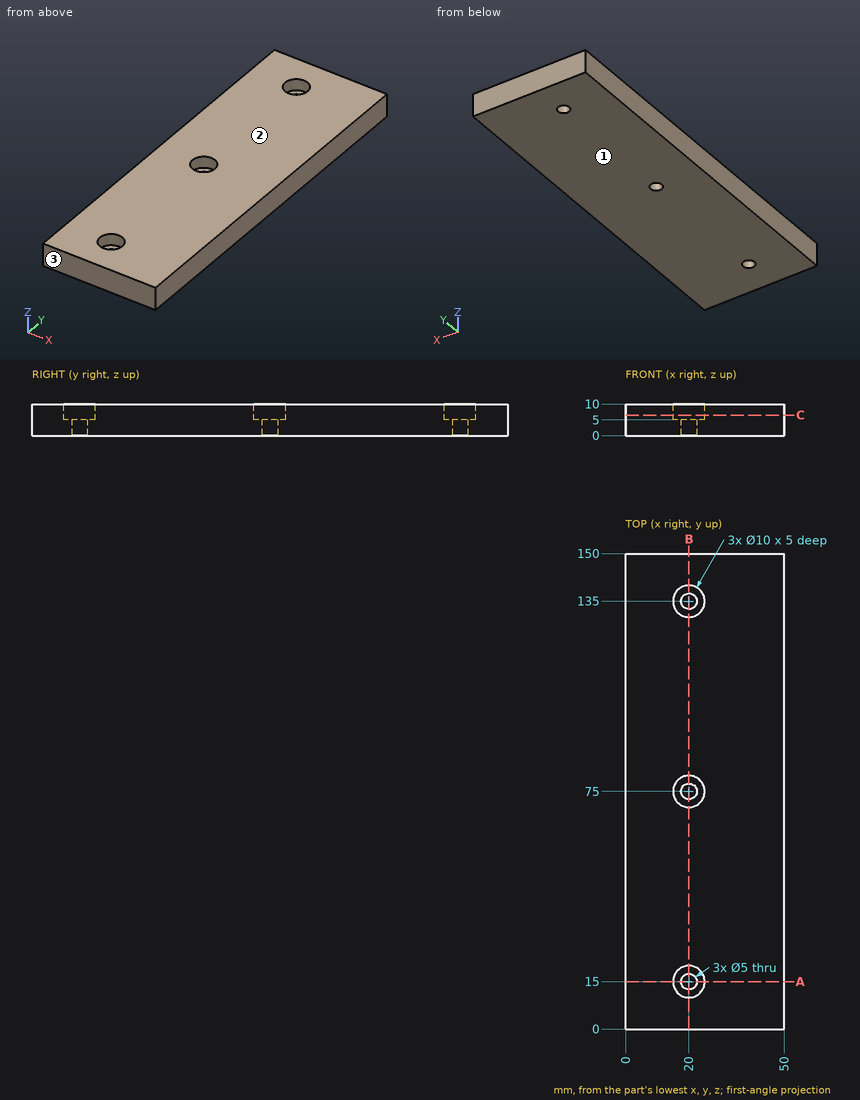
Print and shaded views of the part. All mm, measured from the part's lowest x, y and z. Coordinates: 2 decimals unless noted, no trailing zeros. Order: outer loops, then holes, each group sorted by start corner. A loop starts at its lowest first (then second) coordinate and runs counter-clockwise, first axis right, second up. Notation, with made-up numbers: (49.5, -24) - (78.5, -24) arc R24 ccw to (78.5, 1) - close; hole circle Ø8 at (-32, -37). An arc over 180 degrees is marked (long way). Return JSON: item names as keys, results as strings. Group by question number.
Item 1: Cut at C-C (z = 6.5). List the corners of the cut face in (x, y).
Item 2: Cut at A-A (y = 15). List the corners of the cut face in (x, z).
Item 3: Pin check, flat tip, straight feed: pin 1 (6.5 mm diameter, centred on x = 20, y = 15, fed in from +Z). Stop position of the tip, or through.
Item 4: Cut at B-B (x = 20). List the corners of the cut face in (y, z).
Item 5: Pull direction Z, two halves, no side cores. Call the marked faces 1, 2 and 3: pulls with the +Z half, pulls with the -Z half, needs draft (parallel to the pull), parting line crosses it, or undercut.
Item 6: Drill centre lines: probe 1 along Y at (x, z) = (20, 8.1); probe 2 along Y at (x, z) = (20, 2.5); probe 3 along X at (y, z) = (135, 6.95). Where is each one in solid material? Low to high. Write a range as from..to.
Check values:
{
 "1": {"outline": "(0, 0) - (50, 0) - (50, 150) - (0, 150) - close; hole circle Ø10 at (20, 15); hole circle Ø10 at (20, 75); hole circle Ø10 at (20, 135)"},
 "2": {"outline": "(0, 0) - (17.5, 0) - (17.5, 5) - (15, 5) - (15, 10) - (0, 10) - close; (22.5, 0) - (50, 0) - (50, 10) - (25, 10) - (25, 5) - (22.5, 5) - close"},
 "3": {"pin 1": "stops at z = 5"},
 "4": {"outline": "(0, 0) - (12.5, 0) - (12.5, 5) - (10, 5) - (10, 10) - (0, 10) - close; (17.5, 0) - (72.5, 0) - (72.5, 5) - (70, 5) - (70, 10) - (20, 10) - (20, 5) - (17.5, 5) - close; (77.5, 0) - (132.5, 0) - (132.5, 5) - (130, 5) - (130, 10) - (80, 10) - (80, 5) - (77.5, 5) - close; (137.5, 0) - (150, 0) - (150, 10) - (140, 10) - (140, 5) - (137.5, 5) - close"},
 "5": {"face 1": "pulls with the -Z half", "face 2": "pulls with the +Z half", "face 3": "needs draft"},
 "6": {"probe 1": "y = 0..10, 20..70, 80..130, 140..150", "probe 2": "y = 0..12.5, 17.5..72.5, 77.5..132.5, 137.5..150", "probe 3": "x = 0..15, 25..50"}
}
